Read the model definition and answer for the solid it produces. Units are mm, in the model's axes. A direction names the side the tool comes from. Round coordinates to 2 decimals unless told otherwise and drop trailing zeros. Loops run counter-clockwise (first coordinate to the right, second up) from the corner with the lowest first, then second, coordinate; pieces in that order, holes last. Notation, with made-up numbers: M 86.25,-20.5 L 140.25,-20.5 A24 ccw 140.25,13.5 Z; hole C 27,23.25 d7. An arc over 180 degrees is marked long. Write each question's results on one line, items separated by ' | '.
```python
from build123d import *

# Parameters (mm, degrees)
EXTRUDE_1_DEPTH         = 12
SKETCH_2_R              = 16
CUT_EXTRUDE_2_DEPTH     = 9
SKETCH_3_R              = 14
CUT_EXTRUDE_3_DEPTH     = 8
SKETCH_4_R              = 10
CUT_EXTRUDE_4_DEPTH     = 320.631037291
HOLE_WIZARD_M4_2_D      = 3.3
HOLE_WIZARD_M4_3_D      = 3.3
HOLE_WIZARD_M4_3_DEPTH  = 12.1
HOLE_WIZARD_M4_3_TIP    = 0.991420021
HOLE_WIZARD_M3_1_REACH  = 321.756
HOLE_WIZARD_M3_1_BORE_R = 1.25
SKETCH_17_R             = 12
CUT_EXTRUDE_5_DEPTH     = 320.657629385
SKETCH_18_R             = 8
CUT_EXTRUDE_6_DEPTH     = 320.756157129
HOLE_WIZARD_M5_1_D      = 4.2


with BuildPart() as part:
    # 草图1 → 凸台-拉伸1 (new body)
    with BuildSketch(Plane.XY):
        Polygon((-300, -30), (-300, 0), (300, 0), (300, -30), (300, -110), (-300, -110), align=None)
    extrude(amount=EXTRUDE_1_DEPTH)

    # 草图2 → 切除-拉伸2 (cut)
    with BuildSketch(Plane.XY.offset(12)):
        with Locations(Location((225, -80, 0), (0, 0, 180))):
            Circle(SKETCH_2_R)
        with Locations((-225, -80)):
            Circle(SKETCH_2_R)
    extrude(amount=-CUT_EXTRUDE_2_DEPTH, mode=Mode.SUBTRACT)

    # 草图3 → 切除-拉伸3 (cut)
    with BuildSketch(Plane.XY.offset(12)):
        with Locations((-36, -75)):
            Circle(SKETCH_3_R)
    extrude(amount=-CUT_EXTRUDE_3_DEPTH, mode=Mode.SUBTRACT)

    # 草图4 → 切除-拉伸4 (cut, through all)
    with BuildSketch(Plane.XY.offset(4)):
        with Locations((-36, -75)):
            Circle(SKETCH_4_R)
    extrude(amount=-CUT_EXTRUDE_4_DEPTH, mode=Mode.SUBTRACT)

    # M4 螺纹孔2 (through all)
    with Locations(Plane(origin=(0, 0, 0), x_dir=(-1, 0, 0), z_dir=(0, 0, -1))):
        with Locations((-194, -8.25), (194, -8.25)):
            Hole(HOLE_WIZARD_M4_2_D / 2)

    # M4 螺纹孔3
    with Locations(Plane(origin=(0, -110, 0), x_dir=(-1, 0, 0), z_dir=(0, -1, 0))):
        with Locations((-262, -6), (-92, -6), (92, -6), (262, -6)):
            Hole(HOLE_WIZARD_M4_3_D / 2, depth=HOLE_WIZARD_M4_3_DEPTH)
            with Locations((0, 0, -(HOLE_WIZARD_M4_3_DEPTH + HOLE_WIZARD_M4_3_TIP / 2))):  # 118° drill point
                Cone(0, HOLE_WIZARD_M4_3_D / 2, HOLE_WIZARD_M4_3_TIP, mode=Mode.SUBTRACT)

    # M3 螺纹孔1 bore → M3 螺纹孔1 (cut, up to next)
    with BuildSketch(Plane(origin=(0, -110, 0), x_dir=(-1, 0, 0), z_dir=(0, -1, 0)), mode=Mode.PRIVATE) as hole_wizard_m3_1_sk1:
        with Locations((225, -7)):
            Circle(HOLE_WIZARD_M3_1_BORE_R)
    hole_wizard_m3_1_tool1 = extrude(hole_wizard_m3_1_sk1.sketch, amount=-HOLE_WIZARD_M3_1_REACH, mode=Mode.PRIVATE) & part.part
    # M3 螺纹孔1 bore → M3 螺纹孔1 (cut, up to next)
    with BuildSketch(Plane(origin=(0, -110, 0), x_dir=(-1, 0, 0), z_dir=(0, -1, 0)), mode=Mode.PRIVATE) as hole_wizard_m3_1_sk2:
        with Locations((-225, -7)):
            Circle(HOLE_WIZARD_M3_1_BORE_R)
    hole_wizard_m3_1_tool2 = extrude(hole_wizard_m3_1_sk2.sketch, amount=-HOLE_WIZARD_M3_1_REACH, mode=Mode.PRIVATE) & part.part
    add(hole_wizard_m3_1_tool1.solids().sort_by_distance((-225, -110, 7))[0], mode=Mode.SUBTRACT)
    add(hole_wizard_m3_1_tool2.solids().sort_by_distance((225, -110, 7))[0], mode=Mode.SUBTRACT)

    # 草图17 → 切除-拉伸5 (cut, through all)
    with BuildSketch(Plane.XY.offset(3)):
        with Locations((-225, -80)):
            Circle(SKETCH_17_R)
        with Locations((225, -80)):
            Circle(SKETCH_17_R)
    extrude(amount=-CUT_EXTRUDE_5_DEPTH, mode=Mode.SUBTRACT)

    # 草图18 → 切除-拉伸6 (cut, through all)
    with BuildSketch(Plane.XY.offset(12)):
        with Locations((-225, -35)):
            Circle(SKETCH_18_R)
        with Locations((225, -35)):
            Circle(SKETCH_18_R)
    extrude(amount=-CUT_EXTRUDE_6_DEPTH, mode=Mode.SUBTRACT)

    # M5 螺纹孔1 (through all)
    with Locations(Plane.XY.offset(12)):
        with Locations((245, -35), (205, -35), (-245, -35), (-205, -35)):
            Hole(HOLE_WIZARD_M5_1_D / 2)


solid = part.part
```
1. Find section A-A, the plane x = -36. Give the vertices of the cut face in (y, z).
Completed:
outline: M -110,0 L -85,0 L -85,4 L -89,4 L -89,12 L -110,12 Z; M -65,0 L 0,0 L 0,12 L -61,12 L -61,4 L -65,4 Z
2. Determine the mould class of faces 1 (the face through (4, -110, 6)), 2 (the face through (-46.32, -65.54, 8.06)), 3 (the face through (-300, -54, 6)), 4 (the face through (213.01, -79.47, 1.52)) for opening direction Y: released by +Y, released by -Y, zero draft, split by the parting line, or undercut.
Completed:
face 1: released by -Y | face 2: undercut | face 3: zero draft | face 4: undercut
3. Given P1, Ø1.5, axis at x = -225, z = 7, coming from the -Y side; P2, Ø23, axis at x = -36, y = -75, coming from the +Z side, each flat-ended and moving along its own axis, determine where each tip first touches the part or whether it passes through.
Completed:
P1: stops at y = -64.02 | P2: stops at z = 4
4. Find the intervals of material crossed by L1, parallel to Y at x = -225, z = 0.85; L2, parallel to Y at x = -225, z = 6.75; L3, parallel to X at y = -9, z = 0.5, in increasing order.
Completed:
L1: y = -110 to -92, -68 to -43, -27 to 0 | L2: y = -64 to -43, -27 to 0 | L3: x = -300 to -195.47, -192.53 to 192.53, 195.47 to 300
5. Find section B-B, the plane y = -75. Give the vertices of the cut face in (x, z).
Completed:
outline: M -300,0 L -235.91,0 L -235.91,3 L -240.2,3 L -240.2,12 L -300,12 Z; M -214.09,0 L -46,0 L -46,4 L -50,4 L -50,12 L -209.8,12 L -209.8,3 L -214.09,3 Z; M -26,0 L 214.09,0 L 214.09,3 L 209.8,3 L 209.8,12 L -22,12 L -22,4 L -26,4 Z; M 235.91,0 L 300,0 L 300,12 L 240.2,12 L 240.2,3 L 235.91,3 Z
6. Which of the six approach directions +Z, -Z, +X, -X, +Y, -Y give full straight-line access (tool end or side, diameter ignored) to faces 5 (the face through (-223, -68, 3)), 6 (the face through (4, -54, 0))?
Completed:
face 5: +Z | face 6: -Z, +X, -X, +Y, -Y
